Geometry: final body of the model. Coordinates: model frame, mm. Face numbers are marked on the shaded views. Give positions to 0.01 mm unless a question says otherwise; leave off trailing zeros. Write each loop counter-clockwise with the first axis right and the second up, starting at its lowest first coordinate (ties: lowest second). Pieces come first, ordered by that corner, then holes.
from build123d import *

# Parameters (mm, degrees)
EXTRUDE_1_DEPTH        = 80
CHAMFER_1_SIZE         = 5
HOLE_WIZARD_M8_1_D     = 9
HOLE_WIZARD_M8_1_DEPTH = 15
HOLE_WIZARD_M8_1_TIP   = 2.703872786
HOLE_WIZARD_M12_1_D    = 10.2
PATTERN_LINEAR_1_COUNT = 2
PATTERN_LINEAR_1_PITCH = 40


with BuildPart() as part:
    # 草图1 → 凸台-拉伸1 (new body)
    with BuildSketch(Plane(origin=(0, 0, 0), x_dir=(1, 0, 0), z_dir=(0, 1, 0))):
        Polygon((-22.5, -12.5), (12.5, -12.5), (12.5, 22.5), (22.5, 22.5), (22.5, -22.5), (-22.5, -22.5), align=None)
    extrude(amount=EXTRUDE_1_DEPTH)

    # 倒角1
    chamfer_1_edges = [part.edges().sort_by_distance(p)[0] for p in [
        (-22.5, 80, 17.5),
        (-22.5, 0, 17.5),
        (17.5, 80, -22.5),
        (17.5, 0, -22.5),
    ]]
    chamfer(chamfer_1_edges, length=CHAMFER_1_SIZE)

    # M8 间隙孔1
    with Locations(Plane(origin=(-5, 60, 12.5), x_dir=(-1, 0, 0), z_dir=(0, 0, -1))):
        with Locations((0, 0), (0, -40)):
            Hole(HOLE_WIZARD_M8_1_D / 2, depth=HOLE_WIZARD_M8_1_DEPTH)
            with Locations((0, 0, -(HOLE_WIZARD_M8_1_DEPTH + HOLE_WIZARD_M8_1_TIP / 2))):  # 118° drill point
                Cone(0, HOLE_WIZARD_M8_1_D / 2, HOLE_WIZARD_M8_1_TIP, mode=Mode.SUBTRACT)

    # M12 螺纹孔1 (through all)
    with Locations(Plane(origin=(12.5, 60, -9.5), x_dir=(0, 0, -1), z_dir=(-1, 0, 0))):
        with Locations((0, 0)):
            hole_wizard_m12_1 = Hole(HOLE_WIZARD_M12_1_D / 2)

    # 阵列(线性)1: M12 螺纹孔1 ×2
    with Locations(*[(0, -i * PATTERN_LINEAR_1_PITCH, 0) for i in range(1, PATTERN_LINEAR_1_COUNT)]):
        add(hole_wizard_m12_1, mode=Mode.SUBTRACT)


solid = part.part
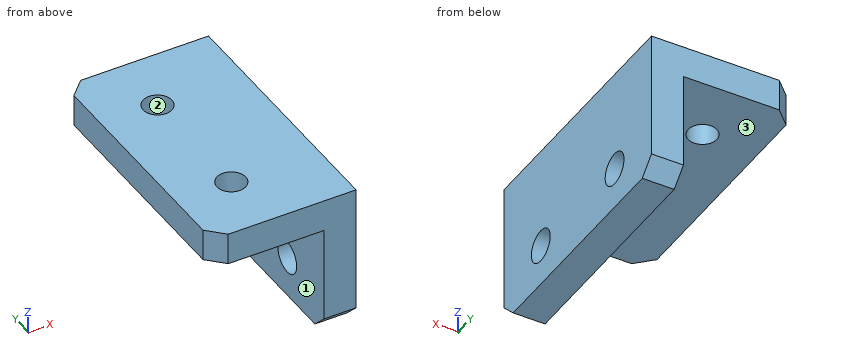
Q1. Section D-D on y = 45. Output: boundary loops of the cut face in (x, z).
Filled sheet:
outline: (-22.5, 12.5) - (12.5, 12.5) - (12.5, -22.5) - (22.5, -22.5) - (22.5, 22.5) - (-22.5, 22.5) - close
Q2. Section B-B on x = -5. Output: boundary loops of the cut face in (y, z).
Filled sheet:
outline: (0, 12.5) - (15.5, 12.5) - (15.5, 22.5) - (0, 22.5) - close; (24.5, 12.5) - (55.5, 12.5) - (55.5, 22.5) - (24.5, 22.5) - close; (64.5, 12.5) - (80, 12.5) - (80, 22.5) - (64.5, 22.5) - close
Q3. Ray query, line 1 along Y through (x, z) = (-5, 19); line 2 along Y through (x, z) = (19, -9.5); line 3 along Z through (x, y) = (20, 20). Return the intervals inside material, ascending.
Filled sheet:
line 1: y = 0 to 15.5, 24.5 to 55.5, 64.5 to 80
line 2: y = 0 to 14.9, 25.1 to 54.9, 65.1 to 80
line 3: z = -22.5 to -14.6, -4.4 to 22.5
Q4. Pin query (flat end, axial travel): P1, Ø12, axis at x = -1, y = 69, coming from the -Z side; P2, Ø16.5, axis at y = 20, z = -9.5, coming from the -X side. Return the tip coordinate at first contact, or that it passes through.
Filled sheet:
P1: stops at z = 12.5
P2: stops at x = 12.5
Q5. Section A-A on y = 60. Output: boundary loops of the cut face in (x, z).
Filled sheet:
outline: (-22.5, 12.5) - (-9.5, 12.5) - (-9.5, 22.5) - (-22.5, 22.5) - close; (-0.5, 12.5) - (12.5, 12.5) - (12.5, -4.4) - (22.5, -4.4) - (22.5, 22.5) - (-0.5, 22.5) - close; (12.5, -22.5) - (22.5, -22.5) - (22.5, -14.6) - (12.5, -14.6) - close
Q6. Pull-direction query (X, two-part tool) for the marked faces 1, 2 and 3; classes: released by +X, released by -X, zero draft, split by the parting line, or undercut.
Filled sheet:
face 1: released by -X
face 2: undercut
face 3: zero draft
Q7. Section C-C on z = -9.5. Output: boundary loops of the cut face in (x, y), plus the area to 3 significant figures.
Filled sheet:
outline: (12.5, 0) - (22.5, 0) - (22.5, 14.9) - (12.5, 14.9) - close; (12.5, 25.1) - (22.5, 25.1) - (22.5, 54.9) - (12.5, 54.9) - close; (12.5, 65.1) - (22.5, 65.1) - (22.5, 80) - (12.5, 80) - close
area: 596 mm2
